Here's how the part is built. I have some questions about the finished solid (model axes, mm). Coordinates: 2 decimals unless noted, no trailing zeros. Order: outer loops, then holes, each group sorted by start corner. A loop starts at its lowest first (then second) coordinate and runs counter-clockwise, first axis right, second up. Notation, with made-up numbers: (11, -19) - (67, -19) arc R22 ccw to (67, 6) - close; hole circle Ø1 at (41.25, 43.5). An arc over 180 degrees is marked (long way). Answer in a Markdown table with one row per item. Add a question column.
Item 1: I want a section at D-D (y = 6.25). Please give me the cut outline in (x, z), plus the area to 3 significant figures.
Item 2: I want a section at A-A (x = 70). Please give me the cut outline in (y, z).
Item 3: I want a section at C-C (y = 0). Please give me the cut outline in (x, z).
Item 4: I want a section at B-B (z = 3.55). Please give me the cut outline in (x, y).
Item 5: If I drill on line 1 along Y through (x, z) = (70, 1.7); line 2 along X through (y, z) = (-2.25, 2.25); line 3 along X through (y, z) = (7, 1.1), over which ranges is the centre line in solid material (lowest first)? Write a range as from..to.
Item 6: Will this pin go through, and if not, where does the flat tip stop? pin 1 Ø8 at (x, y) = (140, 0) entering from +Z.
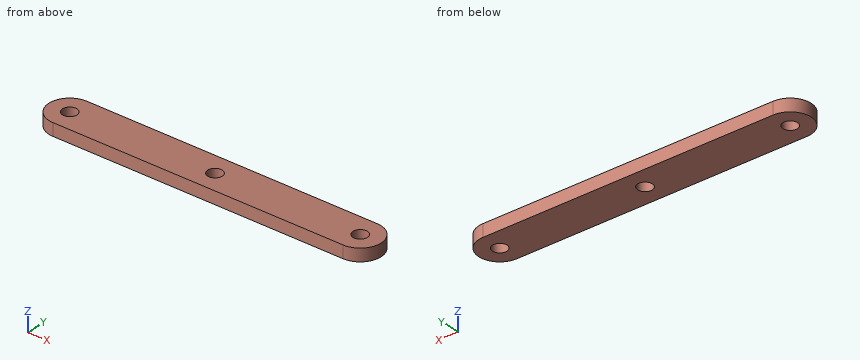
```python
from build123d import *

# Parameters (mm, degrees)
BOSS_EXTRUDE1_DEPTH = 6
SKETCH2_R           = 3.5
CUT_EXTRUDE1_DEPTH  = 95
SKETCH3_R           = 3.5
CUT_EXTRUDE2_DEPTH  = 10


with BuildPart() as part:
    # Sketch1 → Boss-Extrude1 (new body)
    with BuildSketch(Plane.XY):
        with BuildLine():
            Line((0, 10), (140, 10))
            ThreePointArc((140, 10), (150, 0), (140, -10))
            Line((140, -10), (0, -10))
            ThreePointArc((0, -10), (-10, 0), (0, 10))
        make_face()
    extrude(amount=BOSS_EXTRUDE1_DEPTH)

    # Sketch2 → Cut-Extrude1 (cut)
    with BuildSketch(Plane.XY.offset(6)):
        Circle(SKETCH2_R)
        with Locations((140, 0)):
            Circle(SKETCH2_R)
    extrude(amount=-CUT_EXTRUDE1_DEPTH, mode=Mode.SUBTRACT)

    # Sketch3 → Cut-Extrude2 (cut)
    with BuildSketch(Plane.XY.offset(6)):
        with Locations((70, 0)):
            Circle(SKETCH3_R)
    extrude(amount=-CUT_EXTRUDE2_DEPTH, mode=Mode.SUBTRACT)


solid = part.part
```
Values follow:
| question | item | result |
|---|---|---|
| 1 | outline | (-7.81, 0) - (147.81, 0) - (147.81, 6) - (-7.81, 6) - close |
| 1 | area | 934 mm^2 |
| 2 | outline | (-10, 0) - (-3.5, 0) - (-3.5, 6) - (-10, 6) - close; (3.5, 0) - (10, 0) - (10, 6) - (3.5, 6) - close |
| 3 | outline | (-10, 0) - (-3.5, 0) - (-3.5, 6) - (-10, 6) - close; (3.5, 0) - (66.5, 0) - (66.5, 6) - (3.5, 6) - close; (73.5, 0) - (136.5, 0) - (136.5, 6) - (73.5, 6) - close; (143.5, 0) - (150, 0) - (150, 6) - (143.5, 6) - close |
| 4 | outline | (0, -10) - (140, -10) arc R10 ccw to (140, 10) - (0, 10) arc R10 ccw to start; hole circle Ø7 at (0, 0); hole circle Ø7 at (70, 0); hole circle Ø7 at (140, 0) |
| 5 | line 1 | y = -10..-3.5, 3.5..10 |
| 5 | line 2 | x = -9.74..-2.68, 2.68..67.32, 72.68..137.32, 142.68..149.74 |
| 5 | line 3 | x = -7.14..147.14 |
| 6 | pin 1 | stops at z = 6 |
